For this review, use the dimensioned drawing (mm, ordinates from the lowest corner) and the shaded views. Give positions to 0.01 mm unless a question says otherwise; leave off trailing zeros. Order: outer loops, then holes, each group sorted by start corner. A loop starts at its lowest first (then second) coordinate and runs counter-clockwise, first axis right, second up. Notation, with made-up numbers: M 65.5,86.25 L 113.5,86.25 A17 ccw 113.5,90.25 Z; hole C -1.5,18.25 d6. An arc over 180 degrees is marked long. Answer as CSV lines item,"result". Start each with the question number.
1. Clearance check with flat-ended pins moving along their axes: P1, Ø12, axis at y = 52, z = 10.5, coming from the -X side; P2, Ø10, axis at y = 19, z = 8, coming from the +X side; P3, Ø1.5, axis at x = 25, z = 12.5, coming from the +Y side. State where each tip first meets the part, or that it passes through.
2. We need section C-C, the plane z = 9. Give the boundary of the cut face in (x, y).
3. Mouldability with a two-part tool opening along X and no side actions: class the marked faces 1, 2 and 3 as pulls with the +X half, pulls with the -X half, needs draft (parallel to the pull), parting line crosses it, or undercut.
4. We need section A-A, the plane y = 32.5. Give the boundary of the cut face in (x, z), and give its area (3 significant figures).
5. For line 1 along X through (y, z) = (40.5, 43.5); line 2 along Y through (x, z) = (32.5, 22.5); line 3 along X through (y, z) = (28.5, 3), list the stretches that pass through material, from the lowest coordinate up.
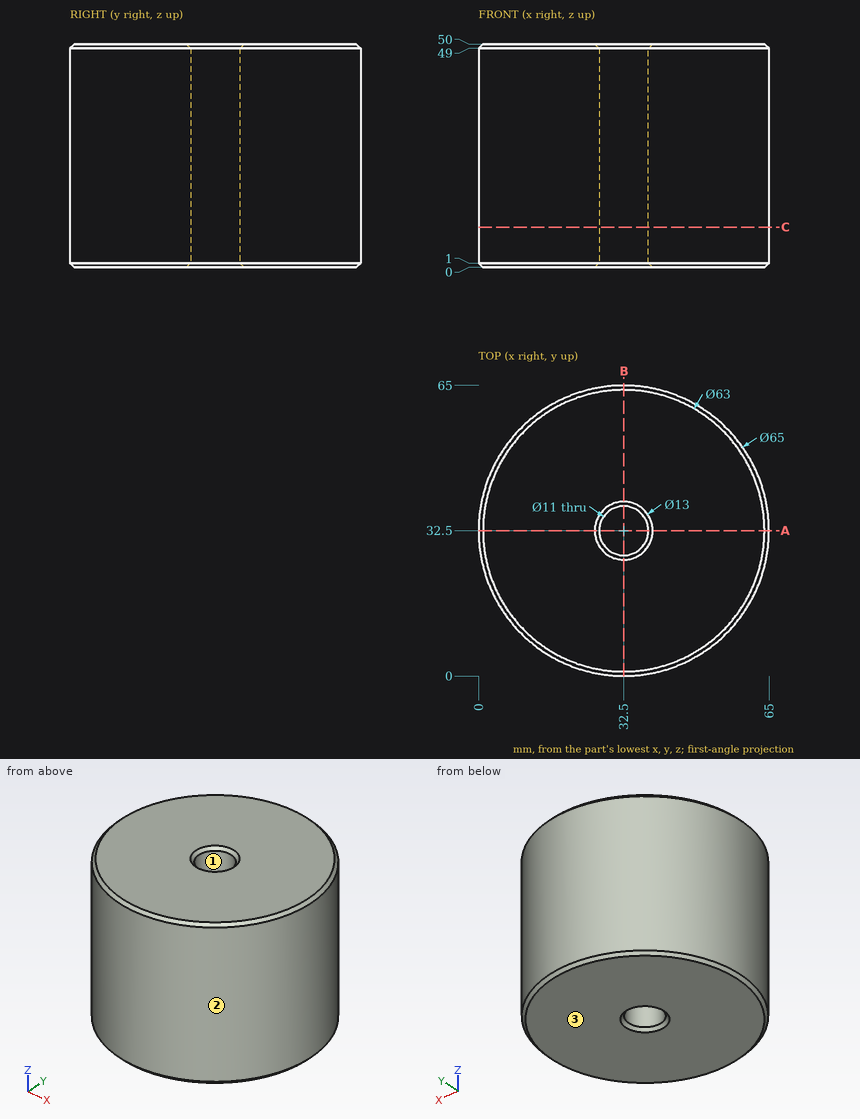
Result set:
1,P1,"x = 2.94"
1,P2,"x = 63.87"
1,P3,"y = 64.29"
2,outline,"C 32.5,32.5 d65; hole C 32.5,32.5 d11"
3,face 1,"undercut"
3,face 2,"parting line crosses it"
3,face 3,"needs draft"
4,outline,"M 0,1 L 1,0 L 26,0 L 27,1 L 27,49 L 26,50 L 1,50 L 0,49 Z; M 38,1 L 39,0 L 64,0 L 65,1 L 65,49 L 64,50 L 39,50 L 38,49 Z"
4,area,"2,700 mm2"
5,line 1,"1 to 64"
5,line 2,"0 to 27, 38 to 65"
5,line 3,"0.25 to 28.73, 36.27 to 64.75"
